from build123d import *

# Parameters (mm, degrees)
SKETCH5_R           = 15
BOSS_EXTRUDE2_DEPTH = 5
BOSS_EXTRUDE3_START = 100
SKETCH6_R           = 15
BOSS_EXTRUDE3_DEPTH = 5
SKETCH7_R           = 17.5
SKETCH7_R_2         = 15
BOSS_EXTRUDE4_DEPTH = 100
SKETCH8_R           = 10
CUT_EXTRUDE1_DEPTH  = 46
BOSS_EXTRUDE5_DEPTH = 20
SKETCH10_R          = 34.5
BOSS_EXTRUDE6_DEPTH = 20
SKETCH11_R          = 10
CUT_EXTRUDE2_DEPTH  = 127
BOSS_EXTRUDE8_REACH = 295.3
FILLET1_R           = 2


with BuildPart() as part:
    # Sketch5 → Boss-Extrude2 (new body)
    with BuildSketch(Plane.XY):
        with BuildLine():
            Line((0, 50), (200, 50))
            ThreePointArc((200, 50), (250, 0), (200, -50))
            Line((200, -50), (0, -50))
            ThreePointArc((0, -50), (-50, 0), (0, 50))
        make_face()
        Circle(SKETCH5_R, mode=Mode.SUBTRACT)
    extrude(amount=BOSS_EXTRUDE2_DEPTH)



with BuildPart() as body_2:
    # Sketch6 → Boss-Extrude3 (new body)
    with BuildSketch(Plane.XY.offset(5).offset(BOSS_EXTRUDE3_START)):
        with BuildLine():
            Line((0, -50), (200, -50))
            ThreePointArc((200, -50), (250, 0), (200, 50))
            Line((200, 50), (0, 50))
            ThreePointArc((0, 50), (-50, 0), (0, -50))
        make_face()
        Circle(SKETCH6_R, mode=Mode.SUBTRACT)
    extrude(amount=BOSS_EXTRUDE3_DEPTH)


with BuildPart() as part_1:
    add(part.part)

    add(body_2.part)  # Boss-Extrude4 merges body 2
    # Sketch7 → Boss-Extrude4 (add)
    with BuildSketch(Plane.XY.offset(5)):
        Circle(SKETCH7_R)
        Circle(SKETCH7_R_2, mode=Mode.SUBTRACT)
    extrude(amount=BOSS_EXTRUDE4_DEPTH)

    # Sketch8 → Cut-Extrude1 (cut)
    with BuildSketch(Plane(origin=(0, 0, 105), x_dir=(-1, 0, 0), z_dir=(0, 0, -1))):
        with Locations((-80, 0)):
            Circle(SKETCH8_R)
        with Locations((-140, 0)):
            Circle(SKETCH8_R)
    extrude(amount=-CUT_EXTRUDE1_DEPTH, mode=Mode.SUBTRACT)

    # Sketch9 → Boss-Extrude5 (add)
    with BuildSketch(Plane.XY.offset(110)):
        with BuildLine():
            Line((80, 35), (140, 35))
            ThreePointArc((140, 35), (175, 0), (140, -35))
            Line((140, -35), (80, -35))
            ThreePointArc((80, -35), (45, 0), (80, 35))
        make_face()
    extrude(amount=BOSS_EXTRUDE5_DEPTH)

    # Sketch10 → Boss-Extrude6 (add)
    with BuildSketch(Plane.XY.offset(130)):
        with Locations((140, 0)):
            Circle(SKETCH10_R)
    extrude(amount=BOSS_EXTRUDE6_DEPTH)

    # Sketch11 → Cut-Extrude2 (cut)
    with BuildSketch(Plane(origin=(0, 0, 0), x_dir=(-1, 0, 0), z_dir=(0, 0, -1))):
        with Locations(Location((-224.307420274, 0, 0), (0, 0, 180))):
            Circle(SKETCH11_R)
    extrude(amount=-CUT_EXTRUDE2_DEPTH, mode=Mode.SUBTRACT)

    # Sketch13 → Boss-Extrude8 (add, up to next)
    with BuildSketch(Plane.XY.offset(5), mode=Mode.PRIVATE) as boss_extrude8_sk1:
        with BuildLine():
            Line((-33.713123493, 36.924589427), (-30.341811144, 33.232130484))
            ThreePointArc((-30.341811144, 33.232130484), (-44.79995187, 4.238432777), (-36.035736887, -26.952285005))
            Line((-36.035736887, -26.952285005), (-40.039707652, -29.946983339))
            ThreePointArc((-40.039707652, -29.946983339), (-49.777724301, 4.709369752), (-33.713123493, 36.924589427))
        make_face()
    boss_extrude8_tool1 = extrude(boss_extrude8_sk1.sketch, amount=BOSS_EXTRUDE8_REACH, mode=Mode.PRIVATE) - part_1.part
    add(boss_extrude8_tool1.solids().sort_by_distance((-32.542205, 34.608391, 5))[0])

    # Fillet1
    fillet1_edges = [part_1.edges().sort_by_distance(p)[0] for p in [
        (105.5, 0, 150),
    ]]
    fillet(fillet1_edges, radius=FILLET1_R)


solid = part_1.part
Verification items for the finished model (mm, model axes). A direction names the side the tool comes from. Coordinates: 2 decimals unless noted, no trailing zeros. Order: outer loops, then holes, each group sorted by start corner. A loop starts at its lowest first (then second) coordinate and runs counter-clockwise, first axis right, second up. Notation, with made-up numbers: (-36, 27) -> (-18, 27) arc R29 cw to (-18, 55) -> close; hole circle Ø4 at (19.25, 62.5). An arc over 180 degrees is marked (long way). Use CSV: the item, a comma, the result in double quotes. Start each with the question number.
Q1. Tool access check on faces 4 (the flat face through (110, 35, 120)), 5 (the flat face through (80, 0, 110)), 6 (the flat face through (110, -35, 120)). Record the directions out of +Z, -Z, +X, -X, +Y, -Y that give a thin tool (end or side, any length) a straight path to the whole face; none if there is none.
Q2. Draft check along Z on faces 1 (the cylindrical face through (-13.887, -10.648, 54.3)), 2 (the cylindrical face through (172.907, 10.363, 138.874)), 3 (the flat face through (82, 0, 130)). Enter one of: +Z half, -Z half, draft (parallel to the pull), parting line (faces both ways), or undercut.
Q3. Section check A-A, the plane z = 43. Record the cut outline in (x, y), and give its area (3 significant figures).
Q4. Depth check by flat-ended pin: P1, Ø10, axis at x = 104, z = 122.5, coming from the +Y side; P2, Ø12, axis at x = 224.31, y = 0, coming from the -Z side; P3, Ø8, axis at y = 36.5, z = 25, coming from the -X side; P4, Ø3, axis at x = 32.5, y = -28, coming from the +Z side. Enter the tip coordinate at first touch or a pass-through.
Q5. Thickness scan on line 1 along Z through (x, y) = (66.5, 11); line 2 along Z through (x, y) = (206, 2); line 3 along Y through (x, z) = (140, 108.35). Record the ranges inside material, lowest first.
Q6. Section check C-C, the plane y = 0. Give the number of separate pieces and of enclosed holes in the cut face, and give its area (3 significant figures).
Q7. Section check B-B, the plane x = 53. Record the cut outline in (y, z), and give its area (3 significant figures).
Returned:
1,face 4,"+Z, +X, -X, +Y"
1,face 5,"none"
1,face 6,"+Z, +X, -X, -Y"
2,face 1,"undercut"
2,face 2,"draft"
2,face 3,"+Z half"
3,outline,"(-40.04, -29.95) -> (-36.04, -26.95) arc R45 cw to (-30.34, 33.23) -> (-33.71, 36.92) arc R50 ccw to start; circle Ø35 at (0, 0); hole circle Ø30 at (0, 0)"
3,area,"605 mm^2"
4,P1,"stops at y = 35"
4,P2,"passes through"
4,P3,"stops at x = -38"
4,P4,"stops at z = 110"
5,line 1,"z = 0 to 5, 105 to 130"
5,line 2,"z = 0 to 5, 105 to 110"
5,line 3,"y = -50 to -10, 10 to 50"
6,separate pieces,"4"
6,enclosed holes,"1"
6,area,"7,280 mm^2"
7,outline,"(-50, 0) -> (50, 0) -> (50, 5) -> (-50, 5) -> close; (-50, 105) -> (50, 105) -> (50, 110) -> (22.27, 110) -> (22.27, 130) -> (-22.27, 130) -> (-22.27, 110) -> (-50, 110) -> close"
7,area,"1,890 mm^2"
